Input: part model. Units: mm. Frame: model coordinates. A direction names the side the tool comes from. Give positions to 0.01 mm unless a question says otherwise; leave off trailing zeros. Write each loop counter-clockwise with the first axis right and the second up, starting at its lowest first coordinate (ties: lowest second). Pieces come first, ordered by that corner, then holes. Notation, with made-up numbers: (-21.5, -3) - (29.5, -3) arc R9 cw to (29.5, 6) - close; hole circle Ø4 at (3, 84.5). An arc over 180 degrees is marked (long way). Use a Markdown table: item, result. Add a question column.
1. Mould query, pull axis X, two halves, no side actions, for faces 3 (the flat face through (-9, 0, -5)), 4 (the cylindrical face through (9.274, 15.783, 2.059)), 5 (the cylindrical face through (12.4, 1.3, -6.5)). Classes: released by +X, released by -X, zero draft, split by the parting line, or undercut.
2. Section query A-A, the plane x = 0. Return loops of the section in (y, z).
3. Section query B-B, the plane z = 0. Return loops of the section in (x, y).
4. Section query C-C, the plane y = 8.5. Return loops of the section in (x, z), plus the area to 3 significant figures.
5. Pin query (flat end, axial travel): pin 1 (1 mm diameter, centred on x = -8.5, y = 3.5, fed in from -Z); pin 2 (10 mm diameter, centred on x = -11, y = 23.5, fed in from -Z); pin 3 (2 mm diameter, centred on x = -4.5, z = 11, fed in from +Y); pin 4 (2 mm diameter, centred on x = 4, z = -10, fed in from +Y). Return the tip coordinate at first contact, or that it passes through.
6. Set-up query: faces 1 (the cylindrical face through (10.74, 16.96, 2.38)), 2 (the flat face through (9, 32, -5)). Return all of +Z, -Z, +X, -X, +Y, -Y with unobstructed straight access to the full face (end or side cutting, diameter ignored); none if empty.
7. Material intervals for probe 1 along X at (y, z) = (17, 0); probe 2 along Z at (x, y) = (2.75, 3.5); probe 3 along X at (y, z) = (6, -2), sorted ascending.
```python
from build123d import *

# Parameters (mm, degrees)
CHAMFER1_SIZE  = 0.5
CHAMFER2_SIZE  = 1
CHAMFER2_SIZE2 = 2


with BuildPart() as part:
    # Sketch1 → Revolve1 (revolve)
    with BuildSketch(Plane.XY, mode=Mode.PRIVATE) as revolve1_sk:
        Polygon((9.5, 0), (14, 0), (14, 2), (11, 2), (11, 32), (9.5, 32), align=None)
    revolve(revolve1_sk.sketch.rotate(Axis((0, 0, 0), (0, 1, 0)), 90), axis=Axis((0, 0, 0), (0, 1, 0)))

    # Chamfer1
    chamfer1_edges = [part.edges().sort_by_distance(p)[0] for p in [
        (0, 32, 9.5),
        (0, 32, 11),
        (0, 2, 14),
        (0, 0, 9.5),
    ]]
    chamfer(chamfer1_edges, length=CHAMFER1_SIZE)

    # Chamfer2
    chamfer2_edges = [part.edges().sort_by_distance(p)[0] for p in [
        (0, 0, 14),
    ]]
    chamfer2_side = [part.faces().sort_by_distance(p)[0] for p in [
        (0, 0.75, 14),
    ]]
    chamfer(chamfer2_edges, length=CHAMFER2_SIZE, length2=CHAMFER2_SIZE2, reference=chamfer2_side[0])


solid = part.part
```
Result sheet:
| question | item | result |
|---|---|---|
| 1 | face 3 | zero draft |
| 1 | face 4 | undercut |
| 1 | face 5 | split by the parting line |
| 2 | outline | (0, -12) - (1, -14) - (1.5, -14) - (2, -13.5) - (2, -11) - (31.5, -11) - (32, -10.5) - (32, -10) - (31.5, -9.5) - (0.5, -9.5) - (0, -10) - close; (0, 10) - (0.5, 9.5) - (31.5, 9.5) - (32, 10) - (32, 10.5) - (31.5, 11) - (2, 11) - (2, 13.5) - (1.5, 14) - (1, 14) - (0, 12) - close |
| 3 | outline | (-14, 1) - (-12, 0) - (-10, 0) - (-9.5, 0.5) - (-9.5, 31.5) - (-10, 32) - (-10.5, 32) - (-11, 31.5) - (-11, 2) - (-13.5, 2) - (-14, 1.5) - close; (9.5, 0.5) - (10, 0) - (12, 0) - (14, 1) - (14, 1.5) - (13.5, 2) - (11, 2) - (11, 31.5) - (10.5, 32) - (10, 32) - (9.5, 31.5) - close |
| 4 | outline | circle Ø22 at (0, 0); hole circle Ø19 at (0, 0) |
| 4 | area | 96.6 mm² |
| 5 | pin 1 | stops at z = -7.55 |
| 5 | pin 2 | stops at z = -9.22 |
| 5 | pin 3 | stops at y = 31.62 |
| 5 | pin 4 | stops at y = 32 |
| 6 | face 1 | +Y |
| 6 | face 2 | +Z, -Z, +X, -X, +Y |
| 7 | probe 1 | x = -11 to -9.5, 9.5 to 11 |
| 7 | probe 2 | z = -10.65 to -9.09, 9.09 to 10.65 |
| 7 | probe 3 | x = -10.82 to -9.29, 9.29 to 10.82 |
